```python
from build123d import *

# Parameters (mm, degrees)
SKETCH3_R           = 5
BOSS_EXTRUDE1_DEPTH = 10


with BuildPart() as part:
    # Sketch3 → Boss-Extrude1 (new body)
    # profile 1 of 6: a face of its own
    with BuildSketch(Plane.XY):
        with BuildLine():
            Line((27.39481576, 680.560432475), (27.230443202, 686.220183409))
            Line((27.230443202, 686.220183409), (13.205751534, 1169.124769421))
            ThreePointArc((13.205751534, 1169.124769421), (2.770474558, 1164.302567957), (-8.590118071, 1166.059146344))
            Line((-8.590118071, 1166.059146344), (-3.095663833, 682.778262513))
            ThreePointArc((-3.095663833, 682.778262513), (11.13008439, 667.653491235), (27.39481576, 680.560432475))
        make_face()
        with Locations((12.242921242, 682.952647962)):
            Circle(SKETCH3_R, mode=Mode.SUBTRACT)
    # profile 2 of 6: a face of its own
    with BuildSketch(Plane.XY):
        with BuildLine():
            ThreePointArc((-8.590118071, 1166.059146344), (2.770474558, 1164.302567957), (13.205751534, 1169.124769421))
            Line((13.205751534, 1169.124769421), (10.388282273, 1266.137157238))
            ThreePointArc((10.388282273, 1266.137157238), (5.346882565, 1267.310168836), (0.186416397, 1267.711735959))
            ThreePointArc((0.186416397, 1267.711735959), (-4.824372475, 1267.355069011), (-9.729431527, 1266.270812525))
            Line((-9.729431527, 1266.270812525), (-8.590118071, 1166.059146344))
        make_face()
        with Locations((0, 1184)):
            Circle(SKETCH3_R, mode=Mode.SUBTRACT)
    # profile 3 of 6: a face of its own
    with BuildSketch(Plane.XY):
        with BuildLine():
            ThreePointArc((0.186416397, 1267.711735959), (5.346882565, 1267.310168836), (10.388282273, 1266.137157238))
            Line((10.388282273, 1266.137157238), (10.197341299, 1272.711724024))
            ThreePointArc((10.197341299, 1272.711724024), (9.983454072, 1274.768905783), (9.35094194, 1276.738086563))
            ThreePointArc((9.35094194, 1276.738086563), (4.804919365, 1277.462611062), (0.208267791, 1277.711712085))
            ThreePointArc((0.208267791, 1277.711712085), (3.736736195, 1276.243392718), (5.197341299, 1272.711724024))
            ThreePointArc((5.197341299, 1272.711724024), (3.729010557, 1269.172329689), (0.186416397, 1267.711735959))
        make_face()
    # profile 4 of 6: a face of its own
    with BuildSketch(Plane.XY):
        with BuildLine():
            ThreePointArc((0.208267791, 1277.711712085), (4.804919365, 1277.462611062), (9.35094194, 1276.738086563))
            ThreePointArc((9.35094194, 1276.738086563), (0.219193138, 1282.711700148), (-8.938575282, 1276.778052618))
            ThreePointArc((-8.938575282, 1276.778052618), (-4.38942912, 1277.482702512), (0.208267791, 1277.711712085))
        make_face()
    # profile 5 of 6: a face of its own
    with BuildSketch(Plane.XY):
        with BuildLine():
            ThreePointArc((-9.729431527, 1266.270812525), (-4.824372475, 1267.355069011), (0.186416397, 1267.711735959))
            ThreePointArc((0.186416397, 1267.711735959), (-4.802646764, 1272.722649721), (0.208267791, 1277.711712085))
            ThreePointArc((0.208267791, 1277.711712085), (-4.38942912, 1277.482702512), (-8.938575282, 1276.778052618))
            ThreePointArc((-8.938575282, 1276.778052618), (-9.584252789, 1274.790285328), (-9.802658701, 1272.711724024))
            Line((-9.802658701, 1272.711724024), (-9.80007392, 1272.484372008))
            Line((-9.80007392, 1272.484372008), (-9.729431527, 1266.270812525))
        make_face()
    # profile 6 of 6: a face of its own
    with BuildSketch(Plane.XY):
        with Locations((0, 1184)):
            Circle(SKETCH3_R)
    extrude(amount=BOSS_EXTRUDE1_DEPTH)


solid = part.part
```
Source: CAD feature listing. Evaluate the final solid. Frame: model axes, mm. Round coordinates to 2 decimals unless told otherwise and drop trailing zeros. Loops run counter-clockwise (first coordinate to the right, second up) from the corner with the lowest first, then second, coordinate; pieces in that order, holes last.
(1) Contact query for flat-ended pins moving along their axis: pin 1 Ø6 at (x, z) = (8.5, 6) entering from +Y; pin 2 Ø2 at (x, z) = (-1.5, 8.5) entering from -Y; pin 3 Ø6 at (y, z) = (800.5, 7) entering from -X; pin 4 Ø8 at (x, y) = (12.24, 682.95) entering from -Z. Output: stop coordinate, or through.
From the geometry:
pin 1: stops at y = 1281.19
pin 2: stops at y = 674.41
pin 3: stops at x = -4.47
pin 4: passes through
(2) Section query B-B (y = 1168.5). Output: boundary loops of the cut face in (x, z).
From the geometry:
outline: (-8.62, 0) - (13.22, 0) - (13.22, 10) - (-8.62, 10) - close
(3) Section query C-C (y = 825.5). Output: boundary loops of the cut face in (x, z).
From the geometry:
outline: (-4.72, 0) - (23.19, 0) - (23.19, 10) - (-4.72, 10) - close
(4) Pull-direction query (Y, two-part tool) for faces 1 (the flat face through (4, 979, 0)), 2 (the cylindrical face through (10.81, 667.68, 4.93)), 3 (the cylindrical face through (11.16, 678.07, 4.93)); classes: +Y half, -Y half, draft (parallel to the pull), parting line (faces both ways), or undercut.
From the geometry:
face 1: draft
face 2: -Y half
face 3: undercut
(5) Material intervals for probe 1 along Y at (x, z) = (3, 1.5); probe 2 along X at (y, z) = (1191, 7.5); probe 3 along X at (y, z) = (1134, 8), sorted ascending.
From the geometry:
probe 1: y = 670.71 to 1268.57, 1276.85 to 1282.31
probe 2: x = -8.87 to 12.57
probe 3: x = -8.23 to 14.23
(6) Section query A-A (z = 4.5). Output: boundary loops of the cut face in (x, y), and give its area (3 significant figures).
From the geometry:
outline: (-9.8, 1272.71) - (-3.1, 682.78) arc R15.34 ccw to (27.39, 680.56) - (10.2, 1272.71) arc R10 ccw to start; hole circle Ø10 at (0.2, 1272.71); hole circle Ø10 at (12.24, 682.95)
area: 15,200 mm2
